```python
from build123d import *

# Parameters (mm, degrees)
EXTRUDE_1_DEPTH          = 20
SHELL_1_T                = -2
CUT_EXTRUDE_1_DEPTH      = 792
CUT_EXTRUDE_1_DEPTH_BACK = 76
SKETCH_2_R               = 2.75
SKETCH_3_R               = 2.75
CUT_EXTRUDE_2_DEPTH      = 10


with BuildPart() as part:
    # 草图1 → 凸台-拉伸1 (new body)
    with BuildSketch(Plane.XY):
        with BuildLine():
            Line((0, 461), (0, 646))
            Line((0, 646), (367, 646))
            Line((367, 646), (367, 0))
            Line((367, 0), (0, 0))
            Line((0, 0), (0, 261))
            ThreePointArc((0, 261), (100, 361), (0, 461))
        make_face()
    extrude(amount=EXTRUDE_1_DEPTH)

    # 抽壳1
    shell_1_openings = [part.faces().sort_by_distance(p)[0] for p in [
        (193.509053572, 320.303646747, 0),
    ]]
    offset(amount=SHELL_1_T, openings=shell_1_openings, kind=Kind.INTERSECTION)

    # 草图2 → 切除-拉伸1 (cut, two sides: drawn at the far end of the back side and taken through both)
    with BuildSketch(Plane(origin=(0, 2, 0), x_dir=(1, 0, 0), z_dir=(0, 1, 0)).offset(-CUT_EXTRUDE_1_DEPTH_BACK)):
        with Locations(Location((353, -9, 0), (0, 0, 90))):
            Circle(SKETCH_2_R)
    extrude(amount=CUT_EXTRUDE_1_DEPTH + CUT_EXTRUDE_1_DEPTH_BACK, mode=Mode.SUBTRACT)

    # 草图3 → 切除-拉伸2 (cut)
    with BuildSketch(Plane(origin=(2, 0, 0), x_dir=(0, 0, -1), z_dir=(1, 0, 0))):
        with Locations((-9, 632)):
            Circle(SKETCH_3_R)
        with Locations((-9, 552)):
            Circle(SKETCH_3_R)
        with Locations((-9, 472)):
            Circle(SKETCH_3_R)
        with Locations((-9, 14)):
            Circle(SKETCH_3_R)
        with Locations((-9, 129)):
            Circle(SKETCH_3_R)
        with Locations((-9, 244)):
            Circle(SKETCH_3_R)
    extrude(amount=-CUT_EXTRUDE_2_DEPTH, mode=Mode.SUBTRACT)


solid = part.part
```
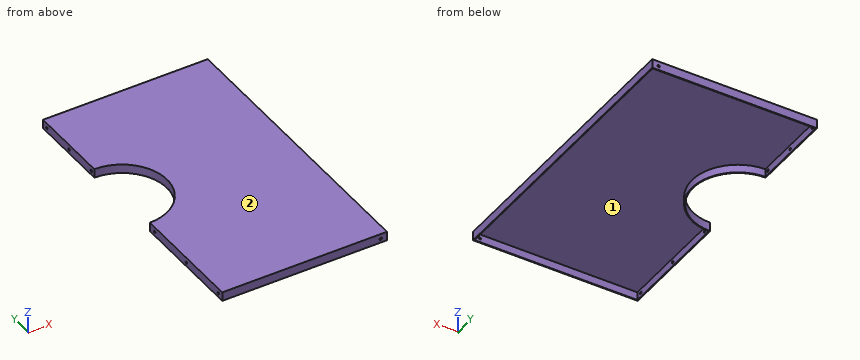
CAD build for the part. Positions are in the model's coordinates, mm. Face numbers are marked on the shaded views. Give positions to 0.01 mm unless a question says otherwise; leave off trailing zeros. Order: outer loops, then holes, each group sorted by start corner. A loop starts at its lowest first (then second) coordinate and runs counter-clockwise, first axis right, second up.
(1) Flat gauge pins, fed straight in: pin 1 (9 mm diameter, centred on x = 126.5, z = 7.5, fed in from -Y); pin 2 (1 mm diameter, centred on y = 313.5, z = 17.5, fed in from -X); pin 3 (3.5 mm diameter, centred on y = 14, z = 9, fed in from -X); pin 4 (1 mm diameter, centred on y = 361.5, z = 8, fed in from -X) (3 decimals). Where does each tip first touch, or does it go through?
(2) Saw through at A-A, the plane y = 76. Give the cut face in (x, z), then the cut area to 3 significant figures.
(3) Drill centre lines: L1, parallel to X at y = 1.35, z = 9; L2, parallel to Z at x = 0.9, y = 472; L3, parallel to Y at x = 227, z = 7.5. Where is each one in solid material? Low to high.
(4) Mould opens along Y. For the marked faces 1 and 2 say: released by +Y, released by -Y, zero draft, split by the parting line, or undercut.
(5) Saw through at B-B, the plane x = 274.5. Give the cut face in (y, z), then the cut area to 3 significant figures.
Results found:
1. pin 1: stops at y = 0
1. pin 2: stops at x = 87.73
1. pin 3: stops at x = 365
1. pin 4: stops at x = 99.995
2. outline: (0, 0) - (2, 0) - (2, 18) - (365, 18) - (365, 0) - (367, 0) - (367, 20) - (0, 20) - close
2. area: 806 mm2
3. L1: x = 0 to 350.25, 355.75 to 367
3. L2: z = 0 to 6.25, 11.75 to 20
3. L3: y = 0 to 2, 644 to 646
4. face 1: undercut
4. face 2: zero draft
5. outline: (0, 0) - (2, 0) - (2, 18) - (644, 18) - (644, 0) - (646, 0) - (646, 20) - (0, 20) - close
5. area: 1,360 mm2
